```python
from build123d import *

# Parameters (mm, degrees)
BOSS_EXTRUDE1_DEPTH = 1062


with BuildPart() as part:
    # Sketch1 → Boss-Extrude1 (new, symmetric)
    with BuildSketch(Plane.XY):
        with BuildLine():
            Line((-50, -90), (-8, -90))
            ThreePointArc((-8, -90), (-2.343145751, -87.656854249), (0, -82))
            Line((0, -82), (0, 82))
            ThreePointArc((0, 82), (-2.343145751, 87.656854249), (-8, 90))
            Line((-8, 90), (-50, 90))
            Line((-50, 90), (-50, 86))
            Line((-50, 86), (-8, 86))
            ThreePointArc((-8, 86), (-5.171572875, 84.828427125), (-4, 82))
            Line((-4, 82), (-4, -82))
            ThreePointArc((-4, -82), (-5.171572875, -84.828427125), (-8, -86))
            Line((-8, -86), (-50, -86))
            Line((-50, -86), (-50, -90))
        make_face()
    extrude(amount=BOSS_EXTRUDE1_DEPTH, both=True)


solid = part.part
```
Geometry check sheet. Reference: the model listing, model coordinates, mm. A direction names the side the tool comes from. Coordinates: 2 decimals unless noted, no trailing zeros. Order: outer loops, then holes, each group sorted by start corner. A loop starts at its lowest first (then second) coordinate and runs counter-clockwise, first axis right, second up. Notation, with made-up numbers: (66, 10.25) - (98, 10.25) arc R4 ccw to (98, 15.25) - close; hole circle Ø5 at (-9, 34.25). An arc over 180 degrees is marked (long way). Answer in a Markdown table with one row per item. Add a question column.
1. Section check C-C (y = -44.5). Enter the section's corners in (x, z).
2. Section check A-A (x = -27). Enter the section's corners in (y, z).
3. Gauge pin test, flat end, axial feed: pin 1 Ø8 at (y, z) = (-67.5, -660) entering from -X. Record the tip position at first contact, or that the pin passes through.
4. Draft check along Y on faces 1 (the face through (-29, -86, 15)), 2 (the face through (-4, 1, 15)), 3 (the face through (0, -1, 15)), 4 (the face through (-29, 90, 15)). Enter one of: +Y half, -Y half, draft (parallel to the pull), parting line (faces both ways), or undercut.
5. Section check B-B (z = 179). Enter the section's corners in (x, y).
6. Material ranges on L1, parallel to Y at x = -9, z = -115.5; L2, parallel to X at y = 5, z = 91; L3, parallel to Y at x = -3, z = 267 (3 decimals), recorded low to high. Write a range as [from, to].
7. Access from +Z, -Z, +X, -X, +Y, -Y to the whole of each face (thin tool, end or side, straight path). Record for faces 5 (the face through (-29, 86, 15)), 6 (the face through (-29, -90, 15)).
Data:
| question | item | result |
|---|---|---|
| 1 | outline | (-4, -1062) - (0, -1062) - (0, 1062) - (-4, 1062) - close |
| 2 | outline | (-90, -1062) - (-86, -1062) - (-86, 1062) - (-90, 1062) - close; (86, -1062) - (90, -1062) - (90, 1062) - (86, 1062) - close |
| 3 | pin 1 | stops at x = -4 |
| 4 | face 1 | undercut |
| 4 | face 2 | undercut |
| 4 | face 3 | draft |
| 4 | face 4 | +Y half |
| 5 | outline | (-50, -90) - (-8, -90) arc R8 ccw to (0, -82) - (0, 82) arc R8 ccw to (-8, 90) - (-50, 90) - (-50, 86) - (-8, 86) arc R4 cw to (-4, 82) - (-4, -82) arc R4 cw to (-8, -86) - (-50, -86) - close |
| 6 | L1 | y = [-90, -86], [86, 90] |
| 6 | L2 | x = [-4, 0] |
| 6 | L3 | y = [-88.245, 88.245] |
| 7 | face 5 | +Z, -Z, -X |
| 7 | face 6 | +Z, -Z, +X, -X, -Y |
